from build123d import *

# Parameters (mm, degrees)
SKETCH_1_W          = 180
SKETCH_1_H          = 80
EXTRUDE_1_DEPTH     = 6
SKETCH_2_R          = 5
CUT_EXTRUDE_1_DEPTH = 6


with BuildPart() as part:
    # 草图1 → 凸台-拉伸1 (new body)
    with BuildSketch(Plane.XY):
        with Locations((90, 40)):
            Rectangle(SKETCH_1_W, SKETCH_1_H)
    extrude(amount=EXTRUDE_1_DEPTH)

    # 草图2 → 切除-拉伸1 (cut)
    with BuildSketch(Plane.XY.offset(6)):
        with Locations((170, 69.998664645)):
            Circle(SKETCH_2_R)
        with Locations((120, 9.998664645)):
            Circle(SKETCH_2_R)
        with Locations((120, 69.998664645)):
            Circle(SKETCH_2_R)
        with Locations((170, 9.998664645)):
            Circle(SKETCH_2_R)
    extrude(amount=-CUT_EXTRUDE_1_DEPTH, mode=Mode.SUBTRACT)


solid = part.part
Can you work these out from the model? Positions are in its coordinate system, mm. Round coordinates to 2 decimals unless told otherwise and drop trailing zeros. Loops run counter-clockwise (first coordinate to the right, second up) from the corner with the lowest first, then second, coordinate; pieces in that order, holes last. Notation, with made-up numbers: (66, 45) - (117, 45) arc R12 ccw to (117, 61) - close; hole circle Ø10 at (23.5, 10). An arc over 180 degrees is marked (long way). Answer in a Markdown table with one row per item. Add a question column.
Q1. We'd pull the mould along Y, two halves only. Please class faces 1 (the cylindrical face through (166, 67, 3)), 2 (the flat face through (89, 80, 3)), 3 (the flat face through (0, 39, 3)): pulls with the +Y half, pulls with the -Y half, needs draft (parallel to the pull), parting line crosses it, or undercut.
Q2. I need wall thicknesses on L1, parallel to Y at x = 120, z = 1.75; L2, parallel to X at y = 10.5, z = 2.05; L3, parallel to X at y = 69, z = 2.75. Which ranges of each line are inside material? Lowest first, please.
Q3. I want a section at C-C on z = 1. List the corners of the cut face in (x, y) for me, and give its area (3 significant figures).
Q4. I want a section at B-B on y = 73. List the corners of the cut face in (x, z) for me.
Q5. I want a section at A-A on x = 120. List the corners of the cut face in (y, z) for me, and give its area (3 significant figures).
Q6. For pin 1 Ø6 at (x, y) = (120, 70) entering from +Z, with a flat end and sliding along its axis, tell me the tip position at first contact or that it passes through.
A:
| question | item | result |
|---|---|---|
| 1 | face 1 | undercut |
| 1 | face 2 | pulls with the +Y half |
| 1 | face 3 | needs draft |
| 2 | L1 | 0 to 5, 15 to 65, 75 to 80 |
| 2 | L2 | 0 to 115.03, 124.97 to 165.03, 174.97 to 180 |
| 2 | L3 | 0 to 115.1, 124.9 to 165.1, 174.9 to 180 |
| 3 | outline | (0, 0) - (180, 0) - (180, 80) - (0, 80) - close; hole circle Ø10 at (120, 10); hole circle Ø10 at (120, 70); hole circle Ø10 at (170, 10); hole circle Ø10 at (170, 70) |
| 3 | area | 14,100 mm^2 |
| 4 | outline | (0, 0) - (116, 0) - (116, 6) - (0, 6) - close; (124, 0) - (166, 0) - (166, 6) - (124, 6) - close; (174, 0) - (180, 0) - (180, 6) - (174, 6) - close |
| 5 | outline | (0, 0) - (5, 0) - (5, 6) - (0, 6) - close; (15, 0) - (65, 0) - (65, 6) - (15, 6) - close; (75, 0) - (80, 0) - (80, 6) - (75, 6) - close |
| 5 | area | 360 mm^2 |
| 6 | pin 1 | through |
